Design review of the part built by this model. Coordinates are the model's own, in mm. A direction names the side the tool comes from. Round coordinates to 2 decimals unless told otherwise and drop trailing zeros. Loops run counter-clockwise (first coordinate to the right, second up) from the corner with the lowest first, then second, coordinate; pieces in that order, holes last. Notation, with made-up numbers: (-30, -2) - (-10, -2) arc R9 ccw to (-10, 10) - close; hole circle Ø2 at (-14, -17). An arc over 180 degrees is marked (long way). Use one line per item in the form item = value. Start each with the question number.
(1) The part is to be moulded in two halves that separate along X. For faces 5 (the cylindrical face through (-74.76, 12.06, -2.17)), 6 (the flat face through (0, 33, 0)), 7 (the flat face through (-15, 40, 15)), 8 (the flat face through (-8, 57, -10)), say which applies: released by +X, released by -X, zero draft, split by the parting line, or undercut.
(2) Wall thickness on probe 1 along X at (y, z) = (13, 0); probe 2 along Y at (x, z) = (-83, 3.5); probe 3 along X at (y, z) = (61.5, -14): over which ranges is each line inside the solid? List them lowest first. Write a range as [from, to].
(3) We need section B-B, the plane z = 0. Write out the cut boundary in (x, y), then the cut area to 3 significant figures.
(4) We need section A-A, the plane x = -65. Write out the cut boundary in (y, z), then the cut area to 3 significant figures.
(5) We need section C-C, the plane y = 59.5. Write out the cut boundary in (x, z), then the cut area to 3 significant figures.
(6) For pin 1 (4.5 mm diameter, centred on x = -9, z = -0.5, fed in from +Y); pin 2 (6 mm diameter, centred on y = 46.5, z = 17.5, fed in from -X); pin 3 (15 mm diameter, centred on x = -75.5, z = 5, fed in from -Y); pin 4 (1 mm diameter, centred on y = 25.5, z = 3.5, fed in from +X), all flat-tipped, find the tip position at first contact; note any pin that passes through.
(7) We need section D-D, the plane x = -9. Write out the cut boundary in (y, z), then the cut area to 3 significant figures.
(8) Machinability: for faces 1 (the flat face through (-24, 26, 5)), 2 (the flat face through (-15, 40, -15)), 3 (the flat face through (-30, 4, 0)), 4 (the flat face through (-56, 16, -6)), which of the approach directions +Z, -Z, +X, -X, +Y, -Y give a long, thin tool a straight path to every point of the face, cutting with its end or side? Answer none if there is none.
from build123d import *

# Parameters (mm, degrees)
ANGLE_BRACKET_BODY_DEPTH      = 25
ANGLE_BRACKET_BODY_DEPTH_BACK = 25
TOP_SLOT_SKETCH_W             = 20
TOP_SLOT_SKETCH_H             = 15
TOP_SLOT_DEPTH                = 15
MOUNTING_HOLE_SKETCH_R        = 10
BASE_MOUNTING_HOLE_DEPTH      = 8
GUSSET_RIB_DEPTH              = 5


with BuildPart() as part:
    # Bracket L-Profile Sketch → Angle Bracket Body (new, two sides: drawn at the far end of the back side and taken through both)
    with BuildSketch(Plane.XY.offset(-ANGLE_BRACKET_BODY_DEPTH_BACK)):
        Polygon((0, 0), (-30, 0), (-30, 8), (-95, 8), (-95, 16), (-15, 16), (-15, 65), (0, 65), align=None)
    extrude(amount=ANGLE_BRACKET_BODY_DEPTH + ANGLE_BRACKET_BODY_DEPTH_BACK)

    # Top Slot Sketch → Top Slot (cut)
    with BuildSketch(Plane.ZY.offset(15)):
        with Locations((0, 57.5)):
            Rectangle(TOP_SLOT_SKETCH_W, TOP_SLOT_SKETCH_H)
    extrude(amount=-TOP_SLOT_DEPTH, mode=Mode.SUBTRACT)

    # Mounting Hole Sketch → Base Mounting Hole (cut)
    with BuildSketch(Plane(origin=(0, 16, 0), x_dir=(1, 0, 0), z_dir=(0, 1, 0))):
        with Locations(Location((-65, 0, 0), (0, 0, 270))):
            Circle(MOUNTING_HOLE_SKETCH_R)
    extrude(amount=-BASE_MOUNTING_HOLE_DEPTH, mode=Mode.SUBTRACT)

    # Gusset Sketch → Gusset Rib (add, symmetric)
    with BuildSketch(Plane.XY):
        Polygon((-15, 50), (-47, 16), (-15, 16), align=None)
    extrude(amount=GUSSET_RIB_DEPTH, both=True)


solid = part.part
Data:
q1.face_5 = undercut
q1.face_6 = released by +X
q1.face_7 = released by -X
q1.face_8 = zero draft
q2.probe_1 = [-95, -75], [-55, 0]
q2.probe_2 = [8, 16]
q2.probe_3 = [-15, 0]
q3.outline = (-95, 8) - (-75, 8) - (-75, 16) - (-95, 16) - close; (-55, 8) - (-30, 8) - (-30, 0) - (0, 0) - (0, 50) - (-15, 50) - (-47, 16) - (-55, 16) - close
q3.area = 1,890 mm^2
q4.outline = (8, -25) - (16, -25) - (16, -10) - (8, -10) - close; (8, 10) - (16, 10) - (16, 25) - (8, 25) - close
q4.area = 240 mm^2
q5.outline = (-15, -25) - (0, -25) - (0, -10) - (-15, -10) - close; (-15, 10) - (0, 10) - (0, 25) - (-15, 25) - close
q5.area = 450 mm^2
q6.pin_1 = 50
q6.pin_2 = -15
q6.pin_3 = 8
q6.pin_4 = 0
q7.outline = (0, -25) - (65, -25) - (65, -10) - (50, -10) - (50, 10) - (65, 10) - (65, 25) - (0, 25) - close
q7.area = 2,950 mm^2
q8.face_1 = +Z, -X, +Y
q8.face_2 = -Z, -X, +Y
q8.face_3 = +Z, -Z, -X, -Y
q8.face_4 = -X, +Y
